The listing builds one solid part. Answer for the finished solid, in the listing's coordinates (mm). Face numbers are marked on the shaded views. A direction names the side the tool comes from. Round coordinates to 2 decimals unless told otherwise and drop trailing zeros. Write each loop counter-clockwise with the first axis right and the second up, starting at its lowest first coordinate (ties: lowest second). Pieces come first, ordered by that corner, then holes. Notation, with made-up numbers: M 47.25,17.25 L 65.25,17.25 A26 ccw 65.25,49.25 Z; hole C 83,-17.75 d9. An arc over 180 degrees is marked long. Write each question's results on one line, items separated by ' | '.
from build123d import *

# Parameters (mm, degrees)
BRACKET_BODY_DEPTH                   = 32.5
TOP_CURVED_SEAT_CUT_R170_DEPTH       = 164.343962239
TOP_CURVED_SEAT_CUT_R170_DEPTH_BACK  = 40
STEP_CURVED_SEAT_CUT_R175_DEPTH      = 12
CURVED_RELIEF_CUT_R115_DEPTH         = 12
CORNER_CHAMFER_CUT_25X30DEG_DEPTH    = 173.771525432
UNDERSIDE_GROOVE_SKETCH_60X30_W      = 30
UNDERSIDE_GROOVE_SKETCH_60X30_H      = 5
UNDERSIDE_GROOVE_60X30X5_DEPTH       = 173.771525432
UNDERSIDE_NOTCH_SKETCH_20X20_W       = 25
UNDERSIDE_NOTCH_SKETCH_20X20_H       = 5
UNDERSIDE_NOTCH_20X20X5_DEPTH        = 192.458219985
C_BORE_HOLE_9_LOW_STEP_D             = 9
C_BORE_HOLE_9_LOW_STEP_CBORE_D       = 20
C_BORE_HOLE_9_LOW_STEP_CBORE_DEPTH   = 25
C_BORE_HOLE_9_HIGH_BLOCK_D           = 9
C_BORE_HOLE_9_HIGH_BLOCK_CBORE_D     = 20
C_BORE_HOLE_9_HIGH_BLOCK_CBORE_DEPTH = 25


with BuildPart() as part:
    # Bracket Side Profile Sketch → Bracket Body (new, symmetric)
    with BuildSketch(Plane.XY):
        Polygon((35, 0), (-125, 0), (-125, 100), (-60, 100), (-60, 60), (-65.09, 60), (-65.09, 48), (-3.45, 48), (-3.45, 36), (35, 36), align=None)
    extrude(amount=BRACKET_BODY_DEPTH, both=True)

    # Top Curved Seat Sketch R170 → Top Curved Seat Cut R170 (cut, two sides: drawn at the far end of the back side and taken through both)
    with BuildSketch(Plane(origin=(0, 100, 0), x_dir=(1, 0, 0), z_dir=(0, 1, 0)).offset(-TOP_CURVED_SEAT_CUT_R170_DEPTH_BACK)):
        with BuildLine():
            ThreePointArc((-60, 32.5), (-63.13553404, 0), (-60, -32.5))
            Line((-60, -32.5), (-60, 32.5))
        make_face()
    extrude(amount=TOP_CURVED_SEAT_CUT_R170_DEPTH + TOP_CURVED_SEAT_CUT_R170_DEPTH_BACK, mode=Mode.SUBTRACT)

    # Step Curved Seat Sketch R175 → Step Curved Seat Cut R175 (cut)
    with BuildSketch(Plane(origin=(0, 48, 0), x_dir=(1, 0, 0), z_dir=(0, 1, 0))):
        with BuildLine():
            ThreePointArc((-65.09, 32.5), (-68.134357932, 0), (-65.09, -32.5))
            Line((-65.09, -32.5), (-65.09, 32.5))
        make_face()
    extrude(amount=STEP_CURVED_SEAT_CUT_R175_DEPTH, mode=Mode.SUBTRACT)

    # Curved Relief Sketch R115 → Curved Relief Cut R115 (cut)
    with BuildSketch(Plane(origin=(0, 36, 0), x_dir=(1, 0, 0), z_dir=(0, 1, 0))):
        with BuildLine():
            Line((-3.45, -32.5), (-3.45, 32.5))
            ThreePointArc((-3.45, 32.5), (-8.137942635, 0), (-3.45, -32.5))
        make_face()
    extrude(amount=CURVED_RELIEF_CUT_R115_DEPTH, mode=Mode.SUBTRACT)

    # Corner Chamfer Sketch 25x30deg → Corner Chamfer Cut 25x30deg (cut, through all)
    with BuildSketch(Plane.XY.offset(32.5)):
        Polygon((-125, 100), (-110.566242501, 100.000001332), (-125, 75), align=None)
    extrude(amount=-CORNER_CHAMFER_CUT_25X30DEG_DEPTH, mode=Mode.SUBTRACT)

    # Underside Groove Sketch 60x30 → Underside Groove 60x30x5 (cut, through all)
    with BuildSketch(Plane.XY.offset(32.5)):
        with Locations((-40, 2.5)):
            Rectangle(UNDERSIDE_GROOVE_SKETCH_60X30_W, UNDERSIDE_GROOVE_SKETCH_60X30_H)
    extrude(amount=-UNDERSIDE_GROOVE_60X30X5_DEPTH, mode=Mode.SUBTRACT)

    # Underside Notch Sketch 20x20 → Underside Notch 20x20x5 (cut, through all)
    with BuildSketch(Plane(origin=(35, 0, 0), x_dir=(0, 0, -1), z_dir=(1, 0, 0))):
        with Locations((0, 2.5)):
            Rectangle(UNDERSIDE_NOTCH_SKETCH_20X20_W, UNDERSIDE_NOTCH_SKETCH_20X20_H)
    extrude(amount=-UNDERSIDE_NOTCH_20X20X5_DEPTH, mode=Mode.SUBTRACT)

    # C-Bore Hole Ø9 Low Step (through all)
    with Locations(Plane(origin=(0, 48, 0), x_dir=(1, 0, 0), z_dir=(0, 1, 0))):
        with Locations((0, 0)):
            CounterBoreHole(C_BORE_HOLE_9_LOW_STEP_D / 2, C_BORE_HOLE_9_LOW_STEP_CBORE_D / 2, C_BORE_HOLE_9_LOW_STEP_CBORE_DEPTH)

    # C-Bore Hole Ø9 High Block (through all)
    with Locations(Plane(origin=(0, 100, 0), x_dir=(1, 0, 0), z_dir=(0, 1, 0))):
        with Locations((-90, 0)):
            CounterBoreHole(C_BORE_HOLE_9_HIGH_BLOCK_D / 2, C_BORE_HOLE_9_HIGH_BLOCK_CBORE_D / 2, C_BORE_HOLE_9_HIGH_BLOCK_CBORE_DEPTH)


solid = part.part
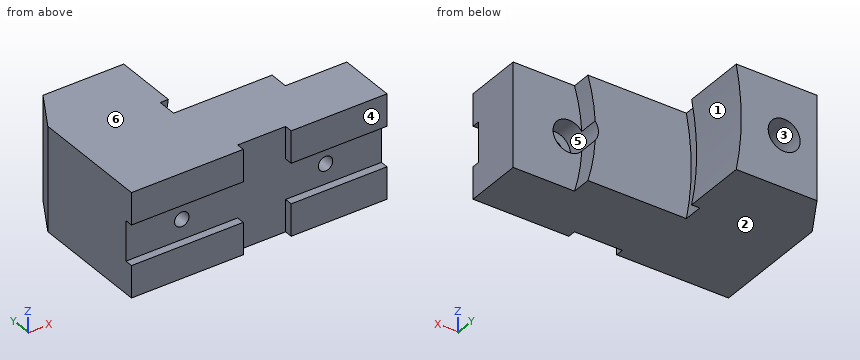
1) The mould has two halves that part along Z. Classify the marked faces 4, 5 and 6: +Z half, -Z half, draft (parallel to the pull), parting line (faces both ways), or undercut.
Return value:
face 4: draft | face 5: undercut | face 6: +Z half
2) Section B-B (z = 0) is taken. Determine the outline of the cut face in (x, y).
Return value:
outline: M -125,5 L -94.5,5 L -94.5,75 L -100,75 L -100,100 L -110.57,100 L -125,75 Z; M -85.5,5 L -4.5,5 L -4.5,23 L -10,23 L -10,48 L -68.13,48 L -68.13,60 L -63.14,60 L -63.14,100 L -80,100 L -80,75 L -85.5,75 Z; M 4.5,5 L 35,5 L 35,36 L 10,36 L 10,23 L 4.5,23 Z
3) A tool of negligible diameter and unlimited length cuts with its end or side. For the marked faces 1, 2 and 3, from which of +Z, -Z, +X, -X, +Y, -Y can it reach the whole face along a straight path? Write none if from no direction.
Return value:
face 1: +X, +Y | face 2: -Z, +X, -X, +Y, -Y | face 3: +Y
4) Section A-A (x = -90) is taken. Determine the outline of the cut face in (y, z).
Return value:
outline: M 0,-32.5 L 100,-32.5 L 100,-10 L 75,-10 L 75,-4.5 L 5,-4.5 L 5,-12.5 L 0,-12.5 Z; M 0,12.5 L 5,12.5 L 5,4.5 L 75,4.5 L 75,10 L 100,10 L 100,32.5 L 0,32.5 Z
5) Find the intervals of material crossed by line 1 (X direction, y = 16, z = -0.5); line 2 (Z direction, x = -89.5, y = 95.5); line 3 (Y direction, x = -47, z = 24), in increasing order.
Return value:
line 1: -125 to -94.47, -85.53 to -4.47, 4.47 to 35 | line 2: -32.5 to -9.99, 9.99 to 32.5 | line 3: 5 to 48
6) Section D-D (x = 0) is taken. Determine the outline of the cut face in (y, z), then the cut area to 3 significant figures.
Return value:
outline: M 0,-32.5 L 36,-32.5 L 36,-10 L 23,-10 L 23,-4.5 L 5,-4.5 L 5,-12.5 L 0,-12.5 Z; M 0,12.5 L 5,12.5 L 5,4.5 L 23,4.5 L 23,10 L 36,10 L 36,32.5 L 0,32.5 Z | area: 1,790 mm²
7) Each of these flat-tipped pins is pushed along its axis until it touches: pin 1 (16 mm diameter, centred on x = -90, z = 0, fed in from +Y); pin 2 (1 mm diameter, centred on y = 77, z = 24, fed in from -X); pin 3 (16 mm diameter, centred on x = 0, z = 0, fed in from -Y); pin 4 (4 mm diameter, centred on x = 16.5, y = 39, fed in from -Z). Where does it stop, or does it pass through?
Return value:
pin 1: y = 75 | pin 2: x = -124.13 | pin 3: y = 5 | pin 4: through
8) Section C-C (y = 41.5) is taken. Determine the outline of the cut face in (x, z).
Return value:
outline: M -125,-32.5 L -3.45,-32.5 A115 cw -7.98,-6.03 A10 cw -7.98,6.03 A115 cw -3.45,32.5 L -125,32.5 Z; hole C -90,0 d9
